Check sheet for the modelled part. Datum: model origin and axes. Units: mm. Face numbers are marked on the shaded views. Give positions to 0.01 mm unless a question says otherwise; leave off trailing zeros. Order: outer loops, then holes, each group sorted by start corner. A loop starts at its lowest first (then second) coordinate and runs counter-clockwise, first axis right, second up. Notation, with made-up numbers: (58, 5.25) -> (73, 5.25) arc R26 cw to (73, 37.25) -> close; hole circle Ø6 at (25.25, -15). An arc over 180 degrees is marked (long way). Write each question's results on one line, items separated by ' | '.
from build123d import *

# Parameters (mm, degrees)
SKETCH1_R           = 3.5
BOSS_EXTRUDE1_DEPTH = 8


with BuildPart() as part:
    # Sketch1 → Boss-Extrude1 (new body)
    with BuildSketch(Plane.XY):
        with BuildLine():
            Line((-5.798172106, 13.421777583), (7.10907715, 5.639148423))
            ThreePointArc((7.10907715, 5.639148423), (9.80078667, 3.06238877), (11.131712033, -0.418075011))
            ThreePointArc((11.131712033, -0.418075011), (17.340118207, -6.010126453), (25.57704331, -7.41312731))
            ThreePointArc((25.57704331, -7.41312731), (34.379390092, -16.99617332), (22.557253019, -22.432454651))
            Line((22.557253019, -22.432454651), (-2.875002754, -8.194359513))
            ThreePointArc((-2.875002754, -8.194359513), (-5.104195022, -7.279113116), (-7.487609197, -6.923710526))
            Line((-7.487609197, -6.923710526), (-27.257727584, -6.38499079))
            ThreePointArc((-27.257727584, -6.38499079), (-40.388886249, 6.936592853), (-27.604263246, 20.591091499))
            Line((-27.604263246, 20.591091499), (-12.841633554, 21.373253968))
            ThreePointArc((-12.841633554, 21.373253968), (-10.053936254, 20.438904782), (-8.658, 17.851313892))
            ThreePointArc((-8.658, 17.851313892), (-7.740710394, 15.305581662), (-5.798172106, 13.421777583))
        make_face()
        Circle(SKETCH1_R, mode=Mode.SUBTRACT)
        with Locations((26.118895321, -15.749708163)):
            Circle(SKETCH1_R, mode=Mode.SUBTRACT)
    extrude(amount=BOSS_EXTRUDE1_DEPTH)


solid = part.part
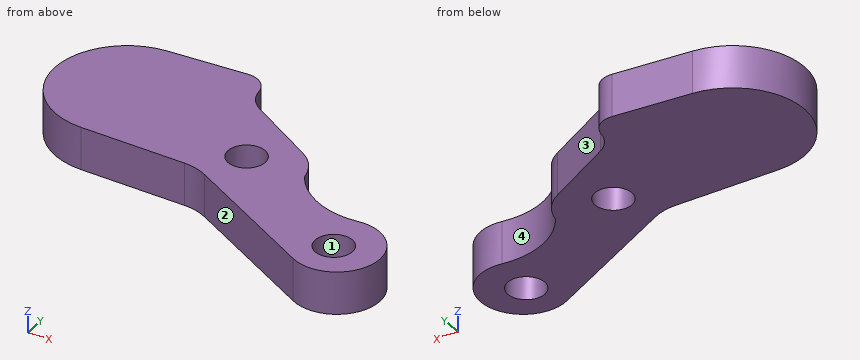
1. Mould release check, pull along X, two halves, no side actions. Record for the marked faces 1, 2, 3 and 4: +X half, -X half, draft (parallel to the pull), parting line (faces both ways), or undercut.
Verdict:
face 1: undercut | face 2: -X half | face 3: +X half | face 4: undercut
2. Section check D-D on x = -15.5. Record the cut outline in (y, z), then the cut area to 3 significant figures.
Verdict:
outline: (-6.71, 0) -> (21.23, 0) -> (21.23, 8) -> (-6.71, 8) -> close | area: 224 mm^2
3. Section check B-B on z = 1. Record the cut outline in (x, y) (3 decimals), then the cut area to 3 significant figures.
Verdict:
outline: (-27.604, 20.591) arc R13.5 ccw to (-27.258, -6.385) -> (-7.488, -6.924) arc R10 cw to (-2.875, -8.194) -> (22.557, -22.432) arc R8.048 ccw (long way) to (25.577, -7.413) arc R15 cw to (11.132, -0.418) arc R8.5 ccw to (7.109, 5.639) -> (-5.798, 13.422) arc R6 cw to (-8.658, 17.851) arc R4 ccw to (-12.842, 21.373) -> close; hole circle Ø7 at (0, 0); hole circle Ø7 at (26.119, -15.75) | area: 1,430 mm^2
4. Section check A-A on x = 1. Record the cut outline in (y, z), then the cut area to 3 significant figures.
Verdict:
outline: (-10.36, 0) -> (-3.35, 0) -> (-3.35, 8) -> (-10.36, 8) -> close; (3.35, 0) -> (9.32, 0) -> (9.32, 8) -> (3.35, 8) -> close | area: 104 mm^2
5. Section check C-C on y = -14.5. Record the cut outline in (x, z), then the cut area to 3 significant figures.
Verdict:
outline: (8.39, 0) -> (22.85, 0) -> (22.85, 8) -> (8.39, 8) -> close; (29.39, 0) -> (34.49, 0) -> (34.49, 8) -> (29.39, 8) -> close | area: 156 mm^2
6. Gauge pin test, flat ends, axial feed: pin 1 Ø4 at (x, z) = (26.5, 4.5) entering from +Y; pin 2 Ø1 at (x, z) = (-8.5, 2.5) entering from -Y; pin 3 Ø1.5 at (x, z) = (-26.5, 3) entering from +Y; pin 4 Ø6.5 at (x, y) = (26.12, -15.75) entering from -Z. Record the tip position at first contact, or that the pin passes through.
Verdict:
pin 1: stops at y = -7.36 | pin 2: stops at y = -6.91 | pin 3: stops at y = 20.69 | pin 4: passes through
7. Material ranges on probe 1 along Y at (x, z) = (27, 4.75); probe 2 along X at (y, z) = (1, 1.75); probe 3 along Y at (x, z) = (0, 5.75), recorded low to high. Write a range as from..to.
Verdict:
probe 1: y = -23.44..-19.14, -12.36..-7.38 | probe 2: x = -38.93..-3.35, 3.35..10.8 | probe 3: y = -9.8..-3.5, 3.5..9.93
